from build123d import *
from OCP.BRepFilletAPI import BRepFilletAPI_MakeChamfer

# Parameters (mm, degrees)
SKETCH1_W           = 8
SKETCH1_H           = 15.5
BOSS_EXTRUDE1_DEPTH = 55
SKETCH2_W           = 5.5
SKETCH2_H           = 11.5
CUT_EXTRUDE1_DEPTH  = 58.699653379
CHAMFER1_SIZE       = 3
CHAMFER1_SIZE2      = 2.517298894
SKETCH3_R           = 1.75
CUT_EXTRUDE2_DEPTH  = 48
SKETCH4_W           = 5.5
SKETCH4_H           = 5
CUT_EXTRUDE3_DEPTH  = 57.756056945
CHAMFER2_SIZE       = 1
CHAMFER2_SIZE2      = 0.839099631


with BuildPart() as part:
    # Sketch1 → Boss-Extrude1 (new body)
    with BuildSketch(Plane(origin=(0, 0, 0), x_dir=(1, 0, 0), z_dir=(0, 1, 0))):
        with Locations((4, 7.75)):
            Rectangle(SKETCH1_W, SKETCH1_H)
    extrude(amount=BOSS_EXTRUDE1_DEPTH)

    # Sketch2 → Cut-Extrude1 (cut, through all)
    with BuildSketch(Plane(origin=(0, 55, 0), x_dir=(1, 0, 0), z_dir=(0, 1, 0))):
        with Locations((2.75, 9.75)):
            Rectangle(SKETCH2_W, SKETCH2_H)
    extrude(amount=-CUT_EXTRUDE1_DEPTH, mode=Mode.SUBTRACT)

    # Chamfer1
    chamfer1_edges = [part.edges().sort_by_distance(p)[0] for p in [
        (0, 27.5, -4),
    ]]
    chamfer1_side = [part.faces().sort_by_distance(p)[0] for p in [
        (0, 27.5, -2),
    ]]
    chamfer(chamfer1_edges, length=CHAMFER1_SIZE, length2=CHAMFER1_SIZE2, reference=chamfer1_side[0])

    # Sketch3 → Cut-Extrude2 (cut)
    with BuildSketch(Plane(origin=(8, 0, 0), x_dir=(0, 0, -1), z_dir=(1, 0, 0))):
        with Locations((11, 50)):
            Circle(SKETCH3_R)
        with Locations((11, 5)):
            Circle(SKETCH3_R)
    extrude(amount=-CUT_EXTRUDE2_DEPTH, mode=Mode.SUBTRACT)

    # Sketch4 → Cut-Extrude3 (cut, through all)
    with BuildSketch(Plane(origin=(0, 0, -4), x_dir=(-1, 0, 0), z_dir=(0, 0, -1))):
        with Locations((-2.75, 52.5)):
            Rectangle(SKETCH4_W, SKETCH4_H)
        with Locations((-2.75, 2.5)):
            Rectangle(SKETCH4_W, SKETCH4_H)
    extrude(amount=-CUT_EXTRUDE3_DEPTH, mode=Mode.SUBTRACT)

    # Chamfer2: one chamfer whose edges measure the first distance from different faces: ONE call of the kernel's chamfer builder (chamfer() names one face for all edges)
    chamfer2_edges_1 = [part.edges().sort_by_distance(p)[0] for p in [
        (6.75, 55, -15.5),
    ]]
    chamfer2_side_1 = [part.faces().sort_by_distance(p)[0] for p in [
        (6.75, 27.5, -15.5),
    ]]
    chamfer2_edges_2 = [part.edges().sort_by_distance(p)[0] for p in [
        (6.75, 0, -15.5),
        (6.75, 0, 0),
    ]]
    chamfer2_side_2 = [part.faces().sort_by_distance(p)[0] for p in [
        (6.75, 0, -7.75),
    ]]
    chamfer2_edges_3 = [part.edges().sort_by_distance(p)[0] for p in [
        (6.75, 55, 0),
    ]]
    chamfer2_side_3 = [part.faces().sort_by_distance(p)[0] for p in [
        (4.178571429, 27.5, 0),
    ]]
    chamfer2 = BRepFilletAPI_MakeChamfer(part.part.solid().wrapped)
    for e in chamfer2_edges_1:
        chamfer2.Add(CHAMFER2_SIZE, CHAMFER2_SIZE2, e.wrapped, chamfer2_side_1[0].wrapped)  # the first distance lies on this face
    for e in chamfer2_edges_2:
        chamfer2.Add(CHAMFER2_SIZE, CHAMFER2_SIZE2, e.wrapped, chamfer2_side_2[0].wrapped)  # the first distance lies on this face
    for e in chamfer2_edges_3:
        chamfer2.Add(CHAMFER2_SIZE, CHAMFER2_SIZE2, e.wrapped, chamfer2_side_3[0].wrapped)  # the first distance lies on this face
    add(Compound.cast(chamfer2.Shape()), mode=Mode.REPLACE)


solid = part.part
The listing builds one solid part. Answer for the finished solid, in the listing's coordinates (mm). A direction names the side the tool comes from. Round coordinates to 2 decimals unless told otherwise and drop trailing zeros. Loops run counter-clockwise (first coordinate to the right, second up) from the corner with the lowest first, then second, coordinate; pieces in that order, holes last. Notation, with made-up numbers: M -15,-31 L 34,-31 A25 ccw 34,-4 Z; hole C -3,-5.5 d3. An arc over 180 degrees is marked long. Return JSON: item names as keys, results as strings.
Q1. Find section C-C, the plane y = 39.5. Determine the outline of the cut face in (x, z), plus the area to 3 significant figures.
Results list:
{"outline": "M 0,-1 L 2.52,-4 L 5.5,-4 L 5.5,-15.5 L 8,-15.5 L 8,0 L 0,0 Z", "area": "57.0 mm2"}
Q2. Which of the six approach directions +Z, -Z, +X, -X, +Y, -Y give full straight-line access (tool end or side, diameter ignored) to faces 1 (the face through (3, 5, -2)), 2 (the face through (4, 28, -4)), 3 (the face through (3, 50, -2))?
Results list:
{"face 1": "+Z, -Z, -X, -Y", "face 2": "-Z, -X, +Y, -Y", "face 3": "+Z, -Z, -X, +Y"}
Q3. Find section B-B, the plane x = 7.5. Determine the outline of the cut face in (y, z), plus the area to 3 significant figures.
Results list:
{"outline": "M 0,-14.5 L 0.84,-15.5 L 54,-15.5 L 55,-14.66 L 55,-0.84 L 54,0 L 0.84,0 L 0,-1 Z; hole C 5,-11 d3.5; hole C 50,-11 d3.5", "area": "832 mm2"}
Q4. The mould has two halves that part along Y. Classify faces 4 (the face through (6.77, 3.45, -11.81)), 5 (the face through (6.73, 54.51, -0.43)), 6 (the face through (7, 0, -8)): released by +Y, released by -Y, zero draft, split by the parting line, or undercut.
Results list:
{"face 4": "undercut", "face 5": "released by +Y", "face 6": "released by -Y"}
Q5. Find section D-D, the plane z = -1.5. Determine the outline of the cut face in (x, y), plus the area to 3 significant figures.
Results list:
{"outline": "M 0.42,5 L 5.5,5 L 5.5,0 L 8,0 L 8,55 L 5.5,55 L 5.5,50 L 0.42,50 Z", "area": "366 mm2"}
Q6. Find section A-A, the plane z = -11. Determine the outline of the cut face in (x, y), plus the area to 3 significant figures.
Results list:
{"outline": "M 5.5,0 L 8,0 L 8,3.25 L 5.5,3.25 Z; M 5.5,6.75 L 8,6.75 L 8,48.25 L 5.5,48.25 Z; M 5.5,51.75 L 8,51.75 L 8,55 L 5.5,55 Z", "area": "120 mm2"}
Q7. Each of these flat-tipped pins is pushed along its axis until it touches: pin 1 Ø4 at (y, z) = (50, -11) entering from -X; pin 2 Ø3 at (x, z) = (2, -1.5) entering from +Y; pin 3 Ø4.5 at (x, z) = (2.5, -2.5) entering from -Y; pin 4 Ø4 at (x, z) = (2, -8.5) entering from +Y. Where does it stop, or does it pass through?
Results list:
{"pin 1": "stops at x = 5.5", "pin 2": "stops at y = 50", "pin 3": "stops at y = 5", "pin 4": "passes through"}
Q8. Find the intervals of material crossed by line 1 along Y through (x, z) = (6.7, -11); line 2 along X through (y, z) = (28, -10); line 3 along Z through (x, y) = (4.75, 24.5), in increasing order. Write a range as from..to.
Results list:
{"line 1": "y = 0..3.25, 6.75..48.25, 51.75..55", "line 2": "x = 5.5..8", "line 3": "z = -4..0"}
